Check sheet for the drawn part. Datum: minimum x, y, z corner. Units: mm. Coordinates: 2 decimals unless noted, no trailing zeros. Write each loop counter-clockwise with the first axis right and the second up, starting at its lowest first coordinate (ties: lowest second). Pieces come first, ordered by that corner, then holes. Notation, with made-up numbers: M 74.5,22.5 L 122.5,22.5 A23 cw 122.5,44.5 Z; hole C 34.5,26 d5. An arc over 180 degrees is marked long. Answer in a Markdown table with one row per item.
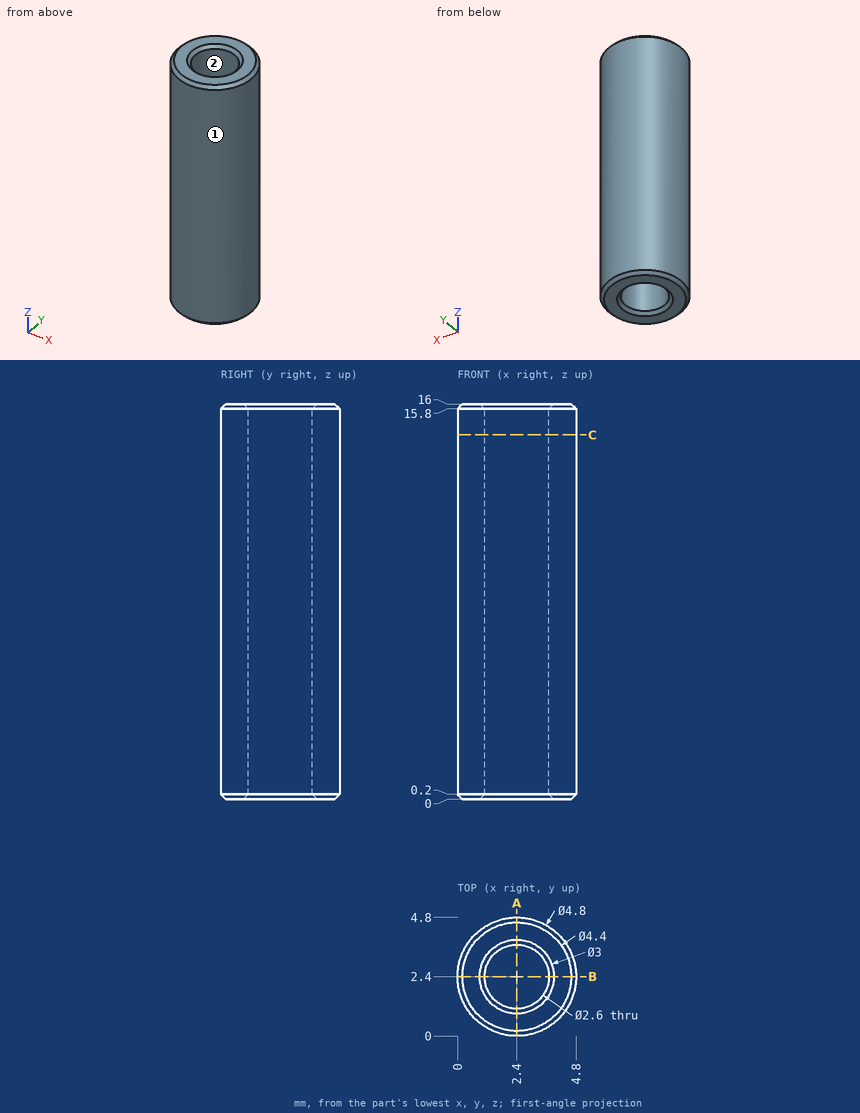
1) Sectioned sample at C-C (z = 14.75). Record the cut outline in (x, y).
Response values:
| item | result |
|---|---|
| outline | C 2.4,2.4 d4.8; hole C 2.4,2.4 d2.6 |
2) Sectioned sample at A-A (x = 2.4). Record the cut outline in (y, z).
Response values:
| item | result |
|---|---|
| outline | M 0,0.2 L 0.2,0 L 0.9,0 L 1.1,0.2 L 1.1,15.8 L 0.9,16 L 0.2,16 L 0,15.8 Z; M 3.7,0.2 L 3.9,0 L 4.6,0 L 4.8,0.2 L 4.8,15.8 L 4.6,16 L 3.9,16 L 3.7,15.8 Z |
3) Release check for a two-part mould opening along X. For the marked faces 1 and 2 record: +X half, -X half, draft (parallel to the pull), parting line (faces both ways), or undercut.
Response values:
| item | result |
|---|---|
| face 1 | parting line |
| face 2 | undercut |
4) Depth check by flat-ended pin: pin 1 (2 mm diameter, centred on y = 4, z = 11.5, fed in from -X). Enter the tip coordinate at first touch or a pass-through.
Response values:
| item | result |
|---|---|
| pin 1 | stops at x = 0.08 |
5) Thickness scan on L1, parallel to Y at x = 2.4, z = 10.75; L2, parallel to Y at x = 3.3, z = 4.75. Record the ranges inside material, lowest first. Write a range as [from, to].
Response values:
| item | result |
|---|---|
| L1 | y = [0, 1.1], [3.7, 4.8] |
| L2 | y = [0.18, 1.46], [3.34, 4.62] |
